from build123d import *

# Parameters (mm, degrees)
SKETCH_1_W              = 100
SKETCH_1_H              = 140
EXTRUDE_1_DEPTH         = 20
HOLE_WIZARD_M10_1_D     = 8.5
HOLE_WIZARD_M10_1_DEPTH = 24.5
HOLE_WIZARD_M10_1_TIP   = 2.553657631
SKETCH_4_R              = 20
CUT_EXTRUDE_1_DEPTH     = 12
SKETCH_5_R              = 17.5
CUT_EXTRUDE_2_DEPTH     = 87.856203002
HOLE_WIZARD_M6_1_D      = 5
HOLE_WIZARD_M6_1_DEPTH  = 15
HOLE_WIZARD_M6_1_TIP    = 1.502151548


with BuildPart() as part:
    # 草图1 → 凸台-拉伸1 (new body)
    with BuildSketch(Plane(origin=(0, 0, 0), x_dir=(0, 0, -1), z_dir=(1, 0, 0))):
        Rectangle(SKETCH_1_W, SKETCH_1_H)
    extrude(amount=EXTRUDE_1_DEPTH)

    # M10 螺纹孔1
    with Locations(Plane(origin=(0, -70, 0), x_dir=(-1, 0, 0), z_dir=(0, -1, 0))):
        with Locations((-10, 30), (-10, -30)):
            Hole(HOLE_WIZARD_M10_1_D / 2, depth=HOLE_WIZARD_M10_1_DEPTH)
            with Locations((0, 0, -(HOLE_WIZARD_M10_1_DEPTH + HOLE_WIZARD_M10_1_TIP / 2))):  # 118° drill point
                Cone(0, HOLE_WIZARD_M10_1_D / 2, HOLE_WIZARD_M10_1_TIP, mode=Mode.SUBTRACT)

    # 草图4 → 切除-拉伸1 (cut)
    with BuildSketch(Plane(origin=(20, 0, 0), x_dir=(0, 0, -1), z_dir=(1, 0, 0))):
        with Locations((0, 30)):
            Circle(SKETCH_4_R)
    extrude(amount=-CUT_EXTRUDE_1_DEPTH, mode=Mode.SUBTRACT)

    # 草图5 → 切除-拉伸2 (cut, through all)
    with BuildSketch(Plane(origin=(8, 0, 0), x_dir=(0, 0, -1), z_dir=(1, 0, 0))):
        with Locations((0, 30)):
            Circle(SKETCH_5_R)
    extrude(amount=-CUT_EXTRUDE_2_DEPTH, mode=Mode.SUBTRACT)

    # M6 螺纹孔1
    with Locations(Plane(origin=(0, 70, 0), x_dir=(1, 0, 0), z_dir=(0, 1, 0))):
        with Locations((10, 30), (10, -30)):
            Hole(HOLE_WIZARD_M6_1_D / 2, depth=HOLE_WIZARD_M6_1_DEPTH)
            with Locations((0, 0, -(HOLE_WIZARD_M6_1_DEPTH + HOLE_WIZARD_M6_1_TIP / 2))):  # 118° drill point
                Cone(0, HOLE_WIZARD_M6_1_D / 2, HOLE_WIZARD_M6_1_TIP, mode=Mode.SUBTRACT)


solid = part.part
Model file for the job. Use its own axes, mm. A direction names the side the tool comes from. Give positions to 0.01 mm unless a question says otherwise; leave off trailing zeros. Loops run counter-clockwise (first coordinate to the right, second up) from the corner with the lowest first, then second, coordinate; pieces in that order, holes last. Notation, with made-up numbers: (-35.75, 81.25) - (-11.75, 81.25) arc R26 cw to (-11.75, 102.25) - close; hole circle Ø8 at (43, 54.25). An arc over 180 degrees is marked (long way). Use one line per item in the form item = value.
(1) Drop flat-ended pins along their axis: P1, Ø4.5, axis at x = 10, z = 30, coming from the +Y side; P2, Ø4, axis at x = 10, z = -30, coming from the +Y side. Give the stop position or say it passes through.
Determined:
P1 = 54.85
P2 = 54.7
(2) Cut at A-A (z = 0). Give the cut face in (x, y), then the cut area to 3 significant figures.
Determined:
outline = (0, -70) - (20, -70) - (20, 10) - (8, 10) - (8, 12.5) - (0, 12.5) - close; (0, 47.5) - (8, 47.5) - (8, 50) - (20, 50) - (20, 70) - (0, 70) - close
area = 2,040 mm^2
(3) Cut at D-D (y = 58). Give the cut face in (x, z).
Determined:
outline = (0, -50) - (20, -50) - (20, 50) - (0, 50) - close; hole circle Ø5 at (10, -30); hole circle Ø5 at (10, 30)
(4) Cut at C-C (y = 30). Give the cut face in (x, z).
Determined:
outline = (0, -50) - (20, -50) - (20, -20) - (8, -20) - (8, -17.5) - (0, -17.5) - close; (0, 17.5) - (8, 17.5) - (8, 20) - (20, 20) - (20, 50) - (0, 50) - close
(5) Pull direction Z, two halves, no side cores. Call faces 1 (the face through (10.33, 62.4, 27.52)), 2 (the face through (10, -1, -50)), 3 (the face through (0, 1, 1)): pulls with the +Z half, pulls with the -Z half, needs draft (parallel to the pull), parting line crosses it, or undercut.
Determined:
face_1 = undercut
face_2 = pulls with the -Z half
face_3 = needs draft
(6) Drill centre lines: L1, parallel to Z at x = 10, y = 62.25; L2, parallel to Z at x = 9.75, y = -62; L3, parallel to Z at x = 13.75, y = 42.5. Where is each one in solid material? Low to high.
Determined:
L1 = -50 to -32.5, -27.5 to 27.5, 32.5 to 50
L2 = -50 to -34.24, -25.76 to 25.76, 34.24 to 50
L3 = -50 to -15.61, 15.61 to 50
(7) 3-axis set-ups, long thin cutter, end or side, ignore diameter. For faces 4 (the face through (8, 12, 0)), 5 (the face through (10, 70, 1)), 6 (the face through (4.06, 47.35, 2.28)), 7 (the face through (10.33, 62.4, -32.48)), 8 (the face through (6.63, -57.58, -27.41)): which of +Z, -Z, +X, -X, +Y, -Y reach the whole face in a straight line?
Determined:
face_4 = +X
face_5 = +Z, -Z, +X, -X, +Y
face_6 = +X, -X
face_7 = +Y
face_8 = -Y
(8) Cut at B-B (x = 3). Give the cut face in (y, z), then the cut area to 3 significant figures.
Determined:
outline = (-70, -50) - (70, -50) - (70, 50) - (-70, 50) - close; hole circle Ø35 at (30, 0)
area = 13,000 mm^2
